Check sheet for the modelled part. Datum: model origin and axes. Units: mm. A direction names the side the tool comes from. Round coordinates to 2 decimals unless told otherwise and drop trailing zeros. Order: outer loops, then holes, each group sorted by start corner. A loop starts at its lowest first (then second) coordinate and runs counter-clockwise, first axis right, second up. Notation, with made-up numbers: M 34,-34.75 L 61,-34.75 A22 cw 61,-0.75 Z; hole C -9,79.25 d3. An arc over 180 degrees is marked long. One line per item, written item: value. Start each with the question number.
(1) Thickness scan on L1, parallel to Z at x = 31.25, y = 443.5; L2, parallel to Y at x = 15, z = 7.5; L3, parallel to Z at x = 34, y = 18. Record the ranges inside material, lowest first.
(2) Release check for a two-part mould opening along Y. For faces 1 (the face through (21, 0, 7)), 2 (the face through (22, 462, 7)), 3 (the face through (13, 150, 7)) record: released by +Y, released by -Y, zero draft, split by the parting line, or undercut.
(3) Cross-section at C-C, the plane y = 408. Enter the section's corners in (x, z).
(4) Cross-section at A-A, the plane x = 8.5. Enter the section's corners in (y, z).
(5) Access from +Z, -Z, +X, -X, +Y, -Y to the whole of each face (thin tool, end or side, straight path). Record for faces 4 (the face through (23.5, 387, 7)), 5 (the face through (0, 442, 6)).
(6) Cross-section at B-B, the plane x = 29.5. Enter the section's corners in (y, z), and give its area (3 significant figures).
(7) Depth check by flat-ended pin: pin 1 Ø7.5 at (y, z) = (88.5, 4.5) entering from -X; pin 2 Ø3 at (y, z) = (18.5, 7.5) entering from +X. Enter the tip coordinate at first touch or a pass-through.
from build123d import *

# Parameters (mm, degrees)
EXTRUDE_1_DEPTH        = 15
CHAMFER_1_SIZE         = 3
HOLE_WIZARD_M6_1_D     = 5
HOLE_WIZARD_M6_1_DEPTH = 17
HOLE_WIZARD_M6_1_TIP   = 1.502151548


with BuildPart() as part:
    # 草图1 → 凸台-拉伸1 (new body)
    with BuildSketch(Plane.XY):
        Polygon((0, 462), (0, 422), (23.5, 422), (23.5, 352), (0, 352), (0, 312), (23.5, 312), (23.5, 150), (0, 150), (0, 110), (23.5, 110), (23.5, 40), (0, 40), (0, 0), (40.5, 0), (40.5, 462), align=None)
    extrude(amount=EXTRUDE_1_DEPTH)

    # 倒角1
    chamfer_1_edges = [part.edges().sort_by_distance(p)[0] for p in [
        (0, 20, 15),
        (0, 110, 7.5),
        (0, 150, 7.5),
        (0, 312, 7.5),
        (0, 352, 7.5),
        (0, 422, 7.5),
        (0, 462, 7.5),
        (0, 0, 7.5),
        (0, 40, 7.5),
        (0, 442, 15),
        (0, 332, 15),
        (0, 130, 15),
    ]]
    chamfer(chamfer_1_edges, length=CHAMFER_1_SIZE)

    # M6 螺纹孔1
    with Locations(Plane(origin=(40.5, 0, 0), x_dir=(0, 0, -1), z_dir=(1, 0, 0))):
        with Locations((-7.5, 443.5), (-7.5, 358.5), (-7.5, 273.5), (-7.5, 188.5), (-7.5, 103.5), (-7.5, 18.5)):
            Hole(HOLE_WIZARD_M6_1_D / 2, depth=HOLE_WIZARD_M6_1_DEPTH)
            with Locations((0, 0, -(HOLE_WIZARD_M6_1_DEPTH + HOLE_WIZARD_M6_1_TIP / 2))):  # 118° drill point
                Cone(0, HOLE_WIZARD_M6_1_D / 2, HOLE_WIZARD_M6_1_TIP, mode=Mode.SUBTRACT)


solid = part.part
Values found:
1. L1: 0 to 5, 10 to 15
1. L2: 0 to 40, 110 to 150, 312 to 352, 422 to 462
1. L3: 0 to 5.05, 9.95 to 15
2. face 1: released by -Y
2. face 2: released by +Y
2. face 3: undercut
3. outline: M 23.5,0 L 40.5,0 L 40.5,15 L 23.5,15 Z
4. outline: M 0,0 L 40,0 L 40,15 L 0,15 Z; M 110,0 L 150,0 L 150,15 L 110,15 Z; M 312,0 L 352,0 L 352,15 L 312,15 Z; M 422,0 L 462,0 L 462,15 L 422,15 Z
5. face 4: +Z, -Z, -X
5. face 5: +Z, -Z, -X, +Y, -Y
6. outline: M 0,0 L 462,0 L 462,15 L 0,15 Z; hole C 18.5,7.5 d5; hole C 103.5,7.5 d5; hole C 188.5,7.5 d5; hole C 273.5,7.5 d5; hole C 358.5,7.5 d5; hole C 443.5,7.5 d5
6. area: 6,810 mm^2
7. pin 1: x = 23.5
7. pin 2: x = 22.9
